Check sheet for the modelled part. Datum: model origin and axes. Units: mm. A direction names the side the tool comes from. Coordinates: 2 decimals unless noted, no trailing zeros. Order: outer loops, then holes, each group sorted by start corner. A loop starts at its lowest first (then second) coordinate and runs counter-clockwise, first axis right, second up. Notation, with made-up numbers: M -33,83.5 L 8,83.5 A17 ccw 8,104.5 Z; hole C -1,-36.5 d3. An arc over 180 degrees is marked long. Answer in a Markdown table with one row per item. Add a question column.
from build123d import *

# Parameters (mm, degrees)
CHAMFER_1_SIZE = 1


with BuildPart() as part:
    # 草图1 → 旋转1 (revolve)
    with BuildSketch(Plane.XY):
        Polygon((134.449619949, -49.868352239), (161.449619949, -49.868352239), (244.449619949, -48.618352239), (272.449619949, -48.618352239), (272.449619949, -42.118352239), (282.449619949, -42.118352239), (282.449619949, -57.118352239), (122.449619949, -57.118352239), (122.449619949, -51.118352239), (131.449619949, -51.118352239), (131.449619949, -52.118352239), (134.449619949, -52.118352239), align=None)
    revolve(axis=Axis((272.449619949, -57.118352239, 0), (-1, 0, 0)))

    # 倒角1
    chamfer_1_edges = [part.edges().sort_by_distance(p)[0] for p in [
        (282.449619949, -72.118352239, 0),
        (272.449619949, -72.118352239, 0),
        (134.449619949, -64.368352239, 0),
    ]]
    chamfer(chamfer_1_edges, length=CHAMFER_1_SIZE)


solid = part.part
1. Section check A-A on x = 163.5. Enter the section's corners in (y, z), then the cut area to 3 significant figures.
2. Set-up check for faces 1 (the cylindrical face through (127.013, -51.395, -1.802)), 2 (the flat face through (282.45, -57, 0)), 3 (the cylindrical face through (132.971, -62.114, -0.22)): record each of +Z, -Z, +X, -X, +Y, -Y from which the full face is reachable in a straight line by a thin tool's end or side.
3. Release check for a two-part mould opening along X. For faces 4 (the cylindrical face through (277.506, -72.104, -0.66)), 5 (the flat face through (122.45, -57, 0)), 6 (the flat face through (131.45, -61, -4)) record: released by +X, released by -X, zero draft, split by the parting line, or undercut.
4. Go/stop test with flat-tipped pins: pin 1 Ø5 at (x, y) = (153.5, -58.5) entering from -Z; pin 2 Ø12 at (x, z) = (240, 0.5) entering from +Y; pin 3 Ø6 at (y, z) = (-65, -10.5) entering from -X. Record where each tip stops, or that it passes through.
5. Scan lines: line 1 (X direction, y = -52, z = -2.25); line 2 (Z direction, x = 274.5, y = -57); line 3 (X direction, y = -66, z = 9). Record each from-to range of solid material in increasing order.
6. Section check B-B on x = 211. Enter the section's corners in (y, z), then the cut area to 3 significant figures.
Result sheet:
| question | item | result |
|---|---|---|
| 1 | outline | C -57.12,0 d14.56 |
| 1 | area | 167 mm^2 |
| 2 | face 1 | -X |
| 2 | face 2 | +Z, -Z, +X, +Y, -Y |
| 2 | face 3 | none |
| 3 | face 4 | zero draft |
| 3 | face 5 | released by -X |
| 3 | face 6 | undercut |
| 4 | pin 1 | z = -7.25 |
| 4 | pin 2 | y = -48.62 |
| 4 | pin 3 | x = 272.45 |
| 5 | line 1 | 122.45 to 131.45, 134.45 to 282.45 |
| 5 | line 2 | -15 to 15 |
| 5 | line 3 | 272.45 to 282.45 |
| 6 | outline | C -57.12,0 d15.99 |
| 6 | area | 201 mm^2 |
